Geometry check sheet. Reference: the model listing, model coordinates, mm. Coordinates: 2 decimals unless noted, no trailing zeros. Loops run counter-clockwise (first coordinate to the right, second up) from the corner with the lowest first, then second, coordinate; pieces in that order, holes last.
from build123d import *

# Parameters (mm, degrees)
SKETCH_1_W                   = 1814
SKETCH_1_H                   = 140
EXTRUDE_1_DEPTH              = 20
CHAMFER_1_SIZE               = 5
HOLE_WIZARD_M6_1_D           = 6.6
HOLE_WIZARD_M6_1_CBORE_D     = 11
HOLE_WIZARD_M6_1_CBORE_DEPTH = 6.8
SKETCH_5_W                   = 420
SKETCH_5_H                   = 80
SKETCH_5_W_2                 = 414
CUT_EXTRUDE_1_DEPTH          = 910.917029185
FILLET_2_R                   = 10
HOLE_WIZARD_M6_1_2_D         = 5
F_5_0MM_1_D                  = 5
F_5_0MM_1_DEPTH              = 15
F_5_0MM_1_TIP                = 1.502151548


with BuildPart() as part:
    # 草图1 → 凸台-拉伸1 (new body)
    with BuildSketch(Plane(origin=(0, 0, 0), x_dir=(1, 0, 0), z_dir=(0, 1, 0))):
        Rectangle(SKETCH_1_W, SKETCH_1_H)
    extrude(amount=EXTRUDE_1_DEPTH)

    # 倒角1
    chamfer_1_edges = [part.edges().sort_by_distance(p)[0] for p in [
        (907, 10, 70),
        (-907, 10, 70),
        (-907, 10, -70),
        (907, 10, -70),
    ]]
    chamfer(chamfer_1_edges, length=CHAMFER_1_SIZE)

    # Hole Wizard M6 _1 (through all)
    with Locations(Plane(origin=(0, 20, 0), x_dir=(1, 0, 0), z_dir=(0, 1, 0))):
        with Locations((267, 50), (797, 50), (797, -50), (267, -50)):
            CounterBoreHole(HOLE_WIZARD_M6_1_D / 2, HOLE_WIZARD_M6_1_CBORE_D / 2, HOLE_WIZARD_M6_1_CBORE_DEPTH)

    # 草图5 → 切除-拉伸1 (cut, through all)
    with BuildSketch(Plane.XZ):
        with Locations((537, 0)):
            Rectangle(SKETCH_5_W, SKETCH_5_H)
        Rectangle(SKETCH_5_W_2, SKETCH_5_H)
        with Locations((-537, 0)):
            Rectangle(SKETCH_5_W, SKETCH_5_H)
    extrude(amount=-CUT_EXTRUDE_1_DEPTH, mode=Mode.SUBTRACT)

    # 圆角2
    fillet_2_edges = [part.edges().sort_by_distance(p)[0] for p in [
        (-747, 10, 40),
        (-327, 10, 40),
        (-327, 10, -40),
        (-747, 10, -40),
        (327, 10, -40),
        (327, 10, 40),
        (747, 10, 40),
        (747, 10, -40),
        (-207, 10, -40),
        (-207, 10, 40),
        (207, 10, 40),
        (207, 10, -40),
    ]]
    fillet(fillet_2_edges, radius=FILLET_2_R)

    # Hole Wizard M6 _1 2 (through all)
    with Locations(Plane(origin=(0, 20, 0), x_dir=(1, 0, 0), z_dir=(0, 1, 0))):
        with Locations((-679.749998444, 56), (-479.749998444, 56), (-279.749998444, 56), (-79.749998444, 56), (120.250001556, 56), (320.250001556, 56), (520.250001556, 56), (720.250001556, 56), (870.250001556, 56), (870.250001556, -56), (720.250001556, -56), (520.250001556, -56), (320.250001556, -56), (120.250001556, -56), (-79.749998444, -56), (-279.749998444, -56), (-479.749998444, -56), (-679.749998444, -56)):
            Hole(HOLE_WIZARD_M6_1_2_D / 2)

    # Ø5.0mm 暗销孔1
    with Locations(Plane(origin=(0, 20, 0), x_dir=(1, 0, 0), z_dir=(0, 1, 0))):
        with Locations((-689.749998444, 56), (860.250001556, -56)):
            Hole(F_5_0MM_1_D / 2, depth=F_5_0MM_1_DEPTH)
            with Locations((0, 0, -(F_5_0MM_1_DEPTH + F_5_0MM_1_TIP / 2))):  # 118° drill point
                Cone(0, F_5_0MM_1_D / 2, F_5_0MM_1_TIP, mode=Mode.SUBTRACT)


solid = part.part
(1) Gauge pin test, flat end, axial feed: pin 1 Ø8.5 at (x, z) = (267, -50) entering from +Y. Record the tip position at first contact, or that the pin passes through.
Findings:
pin 1: stops at y = 13.2
(2) Sectioned sample at B-B on x = -561. Record the cut outline in (y, z).
Findings:
outline: (0, -70) - (20, -70) - (20, -40) - (0, -40) - close; (0, 40) - (20, 40) - (20, 70) - (0, 70) - close
(3) Sectioned sample at A-A on z = -14.5. Record the cut outline in (x, y), and give its area (3 significant figures).
Findings:
outline: (-907, 0) - (-747, 0) - (-747, 20) - (-907, 20) - close; (-327, 0) - (-207, 0) - (-207, 20) - (-327, 20) - close; (207, 0) - (327, 0) - (327, 20) - (207, 20) - close; (747, 0) - (907, 0) - (907, 20) - (747, 20) - close
area: 11,200 mm2
(4) Scan lines: L1, parallel to X at y = 8.5, z = 50; L2, parallel to X at y = 8.75, z = 24.5; L3, parallel to Z at x = 797, y = 8.75. Record each from-to range of solid material in increasing order.
Findings:
L1: x = -907 to 263.7, 270.3 to 793.7, 800.3 to 907
L2: x = -907 to -747, -327 to -207, 207 to 327, 747 to 907
L3: z = -70 to -53.3, -46.7 to 46.7, 53.3 to 70
